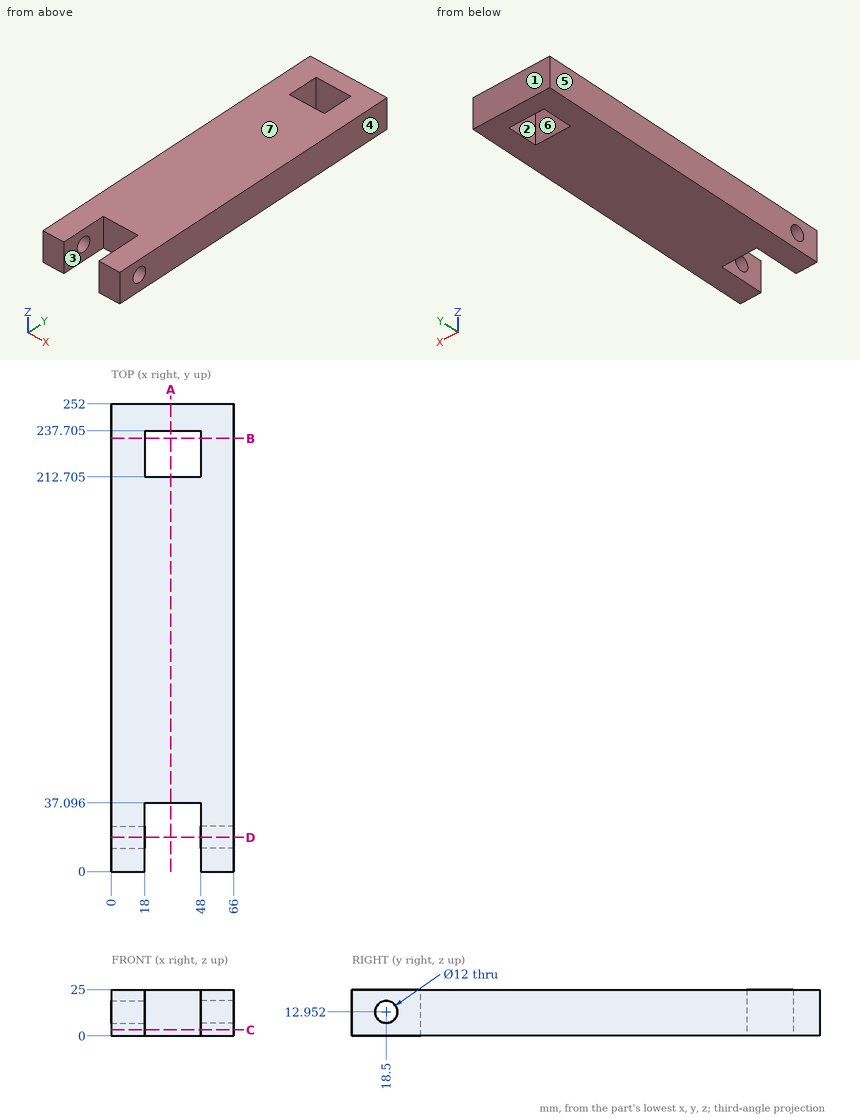
For this review, use the dimensioned drawing (mm, ordinates from the lowest corner) and the shaded views. A direction names the side the tool comes from. Coordinates: 2 decimals unless noted, no trailing zeros. Loops run counter-clockwise (first coordinate to the right, second up) from the corner with the lowest first, then second, coordinate; pieces in that order, holes last.
1. Insertion check: P1, Ø7.5, axis at x = 35.5, z = 14.5, coming from the -Y side. The pin has a flat end and moves straight along its axis. Give the tip position at first contact, or say it passes through.
2. Add section D-D, the plane y = 18.5. Give the boundary of the cut face in (x, z), then the cut area to 3 significant figures.
3. For line 1 (Z direction, x = 53, y = 18); line 2 (Y direction, x = 9, z = 12.25); line 3 (X direction, y = 234, z = 17), list the stretches that pass through material, from the lowest coordinate up.
4. Add section C-C, the plane z = 3.25. Give the boundary of the cut face in (x, y) (1 decimal), then the cut area to 3 significant figures.
5. Mouldability with a two-part tool opening along X and no side actions: class the marked faces 4, 5, 6 and 7 as +X half, -X half, draft (parallel to the pull), parting line (faces both ways), or undercut.
6. Add section A-A, the plane x = 32. Give the boundary of the cut face in (y, z) (1 decimal).
7. For the marked faces 1, 2 and 3, list the 3-axis set-ups (+Z, -Z, +X, -X, +Y, -Y) from which the entire face can be reached by the end or side of a thin tool; tool diameter is ignored.
8. Add section B-B, the plane y = 233.5. Give the boundary of the cut face in (x, z).
Result:
1. P1: stops at y = 37.1
2. outline: (0, 0) - (18, 0) - (18, 6.95) - (0, 6.95) - close; (0, 18.95) - (18, 18.95) - (18, 25) - (0, 25) - close; (48, 0) - (66, 0) - (66, 6.95) - (48, 6.95) - close; (48, 18.95) - (66, 18.95) - (66, 25) - (48, 25) - close
2. area: 468 mm2
3. line 1: z = 0 to 6.97, 18.93 to 25
3. line 2: y = 0 to 12.54, 24.46 to 252
3. line 3: x = 0 to 18, 48 to 66
4. outline: (0, 0) - (18, 0) - (18, 37.1) - (48, 37.1) - (48, 0) - (66, 0) - (66, 252) - (0, 252) - close; hole (18, 212.7) - (48, 212.7) - (48, 237.7) - (18, 237.7) - close
4. area: 14,800 mm2
5. face 4: +X half
5. face 5: -X half
5. face 6: undercut
5. face 7: draft
6. outline: (37.1, 0) - (212.7, 0) - (212.7, 25) - (37.1, 25) - close; (237.7, 0) - (252, 0) - (252, 25) - (237.7, 25) - close
7. face 1: +Z, -Z, +X, -X, +Y
7. face 2: +Z, -Z
7. face 3: +Z, -Z, -Y
8. outline: (0, 0) - (18, 0) - (18, 25) - (0, 25) - close; (48, 0) - (66, 0) - (66, 25) - (48, 25) - close
